Could you check a few things on this model? Use its own coordinates, in mm. Face numbers are marked on the shaded views. Coordinates: 2 decimals unless noted, no trailing zeros. Loops run counter-clockwise (first coordinate to the right, second up) from the corner with the lowest first, then second, coordinate; pieces in that order, holes last. Notation, with made-up numbers: (1, 70) -> (49, 70) arc R22 cw to (49, 80) -> close; hole circle Ø2 at (78.5, -32.5). An arc over 180 degrees is marked (long way). One line per question, with ' | ' between items.
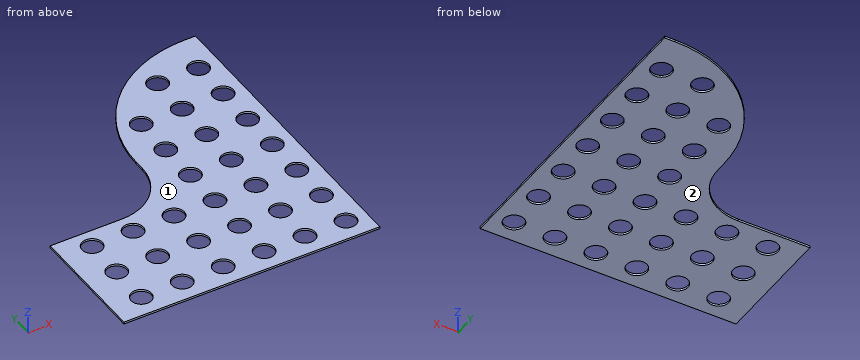
from build123d import *

# Parameters (mm, degrees)
BOSS_EXTRUDE1_DEPTH = 2
SKETCH2_R           = 10
CUT_EXTRUDE1_DEPTH  = 2


with BuildPart() as part:
    # Sketch1 → Boss-Extrude1 (new body)
    with BuildSketch(Plane.XY):
        with BuildLine():
            Line((0, 0), (250, 0))
            Line((250, 0), (250, 300))
            Line((250, 300), (240, 300))
            ThreePointArc((240, 300), (155.147186258, 264.852813742), (120, 180))
            Line((120, 180), (120, 170))
            ThreePointArc((120, 170), (105.355339059, 134.644660941), (70, 120))
            Line((70, 120), (0, 120))
            Line((0, 120), (0, 0))
        make_face()
    extrude(amount=BOSS_EXTRUDE1_DEPTH)

    # Sketch2 → Cut-Extrude1 (cut)
    with BuildSketch(Plane.XY.offset(2)):
        with Locations((230, 261.698838223)):
            Circle(SKETCH2_R)
        with Locations((190, 261.698838223)):
            Circle(SKETCH2_R)
        with Locations((230, 221.698838223)):
            Circle(SKETCH2_R)
        with Locations((190, 221.698838223)):
            Circle(SKETCH2_R)
        with Locations((230, 181.698838223)):
            Circle(SKETCH2_R)
        with Locations((190, 181.698838223)):
            Circle(SKETCH2_R)
        with Locations((230, 141.698838223)):
            Circle(SKETCH2_R)
        with Locations((190, 141.698838223)):
            Circle(SKETCH2_R)
        with Locations((230, 101.698838223)):
            Circle(SKETCH2_R)
        with Locations((190, 101.698838223)):
            Circle(SKETCH2_R)
        with Locations((230, 61.698838223)):
            Circle(SKETCH2_R)
        with Locations((190, 61.698838223)):
            Circle(SKETCH2_R)
        with Locations((230, 21.698838223)):
            Circle(SKETCH2_R)
        with Locations((190, 21.698838223)):
            Circle(SKETCH2_R)
        with Locations((150, 221.698838223)):
            Circle(SKETCH2_R)
        with Locations((150, 181.698838223)):
            Circle(SKETCH2_R)
        with Locations((150, 141.698838223)):
            Circle(SKETCH2_R)
        with Locations((150, 101.698838223)):
            Circle(SKETCH2_R)
        with Locations((150, 61.698838223)):
            Circle(SKETCH2_R)
        with Locations((150, 21.698838223)):
            Circle(SKETCH2_R)
        with Locations((110, 101.698838223)):
            Circle(SKETCH2_R)
        with Locations((70, 101.698838223)):
            Circle(SKETCH2_R)
        with Locations((30, 101.698838223)):
            Circle(SKETCH2_R)
        with Locations((110, 61.698838223)):
            Circle(SKETCH2_R)
        with Locations((70, 61.698838223)):
            Circle(SKETCH2_R)
        with Locations((30, 61.698838223)):
            Circle(SKETCH2_R)
        with Locations((110, 21.698838223)):
            Circle(SKETCH2_R)
        with Locations((70, 21.698838223)):
            Circle(SKETCH2_R)
        with Locations((30, 21.698838223)):
            Circle(SKETCH2_R)
    extrude(amount=-CUT_EXTRUDE1_DEPTH, mode=Mode.SUBTRACT)


solid = part.part
1) If we section it at B-B on x = 155: Please give me the cut outline in (y, z), and give its area (3 significant figures).
Data:
outline: (0, 0) -> (13.04, 0) -> (13.04, 2) -> (0, 2) -> close; (30.36, 0) -> (53.04, 0) -> (53.04, 2) -> (30.36, 2) -> close; (70.36, 0) -> (93.04, 0) -> (93.04, 2) -> (70.36, 2) -> close; (110.36, 0) -> (133.04, 0) -> (133.04, 2) -> (110.36, 2) -> close; (150.36, 0) -> (173.04, 0) -> (173.04, 2) -> (150.36, 2) -> close; (190.36, 0) -> (213.04, 0) -> (213.04, 2) -> (190.36, 2) -> close; (230.36, 0) -> (264.71, 0) -> (264.71, 2) -> (230.36, 2) -> close | area: 322 mm²
2) If we section it at D-D on x = 190: Give the number of separate pieces and of enclosed holes in the cut face, and give its area (3 significant figures).
Data:
separate pieces: 8 | enclosed holes: 0 | area: 298 mm²
3) I need wall thicknesses on line 1 along Y through (x, z) = (110, 0.95); line 2 along X through (y, z) = (133, 1.9); line 3 along X through (y, z) = (190, 0.35). Which ranges of each line are inside material? Lowest first, please. Write a range as from..to.
Data:
line 1: 0..11.7, 31.7..51.7, 71.7..91.7, 111.7..140 | line 2: 103.63..145.07, 154.93..185.07, 194.93..225.07, 234.93..250 | line 3: 120.42..144.42, 155.58..184.42, 195.58..224.42, 235.58..250
4) If we section it at A-A on x = 30: Please give me the cut outline in (y, z).
Data:
outline: (0, 0) -> (11.7, 0) -> (11.7, 2) -> (0, 2) -> close; (31.7, 0) -> (51.7, 0) -> (51.7, 2) -> (31.7, 2) -> close; (71.7, 0) -> (91.7, 0) -> (91.7, 2) -> (71.7, 2) -> close; (111.7, 0) -> (120, 0) -> (120, 2) -> (111.7, 2) -> close
5) We'd pull the mould along Z, two halves only. Please class the marked faces 1 and 2: pulls with the +Z half, pulls with the -Z half, needs draft (parallel to the pull), parting line crosses it, or undercut.
Data:
face 1: pulls with the +Z half | face 2: pulls with the -Z half
6) I'm going to push a flat-ended pin straight in: pin 1 Ø1 at (y, z) = (130.5, 1.5) entering from -X. Where does the tip first touch, or does it pass through?
Data:
pin 1: x = 100
7) If we section it at C-C on y = 225.5: Please give me the cut outline in (x, z).
Data:
outline: (128.96, 0) -> (140.75, 0) -> (140.75, 2) -> (128.96, 2) -> close; (159.25, 0) -> (180.75, 0) -> (180.75, 2) -> (159.25, 2) -> close; (199.25, 0) -> (220.75, 0) -> (220.75, 2) -> (199.25, 2) -> close; (239.25, 0) -> (250, 0) -> (250, 2) -> (239.25, 2) -> close
